```python
from build123d import *

# Parameters (mm, degrees)
SPANNER_BODY_2_5MM_DEPTH       = 2.5
HANDLE_SLOT_RECESS_0_5MM_DEPTH = 0.5


with BuildPart() as part:
    # Spanner Outline Sketch → Spanner Body 2.5mm (new body)
    with BuildSketch(Plane.XY):
        with BuildLine():
            Line((8.874119675, -4.5), (63.125880325, -4.5))
            ThreePointArc((63.125880325, -4.5), (64.96037879, -4.848697453), (66.539003277, -5.846153846))
            ThreePointArc((66.539003277, -5.846153846), (80, 0), (66.539003277, 5.846153846))
            ThreePointArc((66.539003277, 5.846153846), (64.96037879, 4.848697453), (63.125880325, 4.5))
            Line((63.125880325, 4.5), (8.874119675, 4.5))
            ThreePointArc((8.874119675, 4.5), (7.03962121, 4.848697453), (5.460996723, 5.846153846))
            ThreePointArc((5.460996723, 5.846153846), (-3.444494595, 7.220488694), (-7.979967897, -0.565784729))
            Line((-7.979967897, -0.565784729), (-1.75, 3.031088913))
            ThreePointArc((-1.75, 3.031088913), (3.031088913, 1.75), (1.75, -3.031088913))
            Line((1.75, -3.031088913), (-4.479967897, -6.627962556))
            ThreePointArc((-4.479967897, -6.627962556), (0.627224524, -7.975373935), (5.460996723, -5.846153846))
            ThreePointArc((5.460996723, -5.846153846), (7.03962121, -4.848697453), (8.874119675, -4.5))
        make_face()
        Polygon((75.5, -2.020725942), (75.5, 2.020725942), (72, 4.041451884), (68.5, 2.020725942), (68.5, -2.020725942), (72, -4.041451884), align=None, mode=Mode.SUBTRACT)
    extrude(amount=SPANNER_BODY_2_5MM_DEPTH)

    # Handle Slot Sketch → Handle Slot Recess 0.5mm (cut)
    with BuildSketch(Plane.XY.offset(2.5)):
        with BuildLine():
            Line((22, 1.71110999), (50, 1.71110999))
            ThreePointArc((50, 1.71110999), (51.71110999, 0), (50, -1.71110999))
            Line((50, -1.71110999), (22, -1.71110999))
            ThreePointArc((22, -1.71110999), (20.28889001, 0), (22, 1.71110999))
        make_face()
    extrude(amount=-HANDLE_SLOT_RECESS_0_5MM_DEPTH, mode=Mode.SUBTRACT)


solid = part.part
```
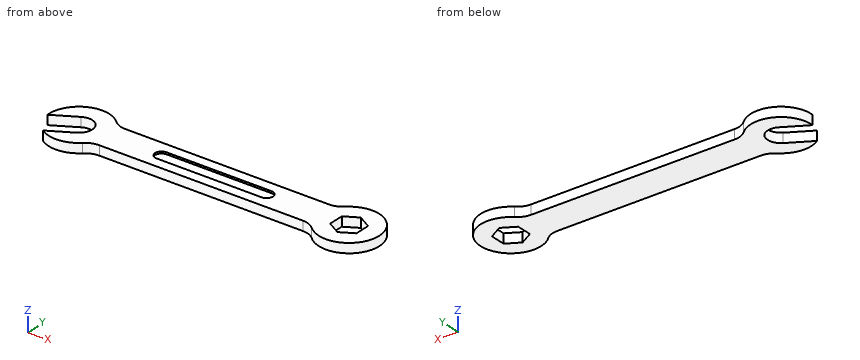
Geometry check sheet. Reference: the model listing, model coordinates, mm. Coordinates: 2 decimals unless noted, no trailing zeros. Loops run counter-clockwise (first coordinate to the right, second up) from the corner with the lowest first, then second, coordinate; pieces in that order, holes last. Notation, with made-up numbers: (-38, 54) - (-30, 54) arc R11 cw to (-30, 70) - close; hole circle Ø2 at (19.5, 39). An arc over 180 degrees is marked (long way). One line per item, written item: value. Start each with the question number.
(1) Depth check by flat-ended pin: P1, Ø1.5, axis at x = 45.5, z = 0.5, coming from the +Y side; P2, Ø1.5, axis at x = 51, z = 2, coming from the -Y side. Enter the tip coordinate at first touch or a pass-through.
(2) Cross-section at D-D on x = 53.5. Enter the section's corners in (y, z).
(3) Cross-section at B-B on z = 0.85. Enter the section's corners in (x, y), plus the area to 3 significant figures.
(4) Cross-section at A-A on x = 0. Enter the section's corners in (y, z).
(5) Material ranges on line 1 (X direction, y = -0.25, z = 1.6); line 2 (X direction, y = 2.25, z = 1.8); line 3 (Y direction, x = 23, z = 2.4), recorded low to high. Write a range as [from, to].
(6) Cross-section at C-C on y = 0.5. Enter the section's corners in (x, z), plus the area to 3 significant figures.
Results below:
1. P1: stops at y = 4.5
1. P2: stops at y = -4.5
2. outline: (-4.5, 0) - (4.5, 0) - (4.5, 2.5) - (-4.5, 2.5) - close
3. outline: (-7.98, -0.57) - (-1.75, 3.03) arc R3.5 cw to (1.75, -3.03) - (-4.48, -6.63) arc R8 ccw to (5.46, -5.85) arc R5 cw to (8.87, -4.5) - (63.13, -4.5) arc R5 cw to (66.54, -5.85) arc R8 ccw (long way) to (66.54, 5.85) arc R5 cw to (63.13, 4.5) - (8.87, 4.5) arc R5 cw to (5.46, 5.85) arc R8 ccw to start; hole (68.5, -2.02) - (72, -4.04) - (75.5, -2.02) - (75.5, 2.02) - (72, 4.04) - (68.5, 2.02) - close
3. area: 801 mm2
4. outline: (-8, 0) - (-4.04, 0) - (-4.04, 2.5) - (-8, 2.5) - close; (3.5, 0) - (8, 0) - (8, 2.5) - (3.5, 2.5) - close
5. line 1: x = [-8, -7.43], [3.49, 68.5], [75.5, 80]
5. line 2: x = [-7.68, -3.1], [2.68, 68.9], [75.1, 79.68]
5. line 3: y = [-4.5, -1.71], [1.71, 4.5]
6. outline: (-7.98, 0) - (-6.13, 0) - (-6.13, 2.5) - (-7.98, 2.5) - close; (3.46, 0) - (68.5, 0) - (68.5, 2.5) - (51.64, 2.5) - (51.64, 2) - (20.36, 2) - (20.36, 2.5) - (3.46, 2.5) - close; (75.5, 0) - (79.98, 0) - (79.98, 2.5) - (75.5, 2.5) - close
6. area: 163 mm2
